from build123d import *

# Parameters (mm, degrees)
SKETCH_1_R      = 12
SKETCH_1_R_2    = 8
EXTRUDE_1_DEPTH = 6
SKETCH_2_W      = 18
SKETCH_2_H      = 2
EXTRUDE_2_DEPTH = 12


with BuildPart() as part:
    # 草图1 → 凸台-拉伸1 (new, symmetric)
    with BuildSketch(Plane.XY):
        Circle(SKETCH_1_R)
        Circle(SKETCH_1_R_2, mode=Mode.SUBTRACT)
    extrude(amount=EXTRUDE_1_DEPTH, both=True)

    # 草图2 → 凸台-拉伸2 (add)
    with BuildSketch(Plane.XY.offset(6)):
        with Locations((20.958260743, 0)):
            Rectangle(SKETCH_2_W, SKETCH_2_H)
    extrude(amount=-EXTRUDE_2_DEPTH)


solid = part.part
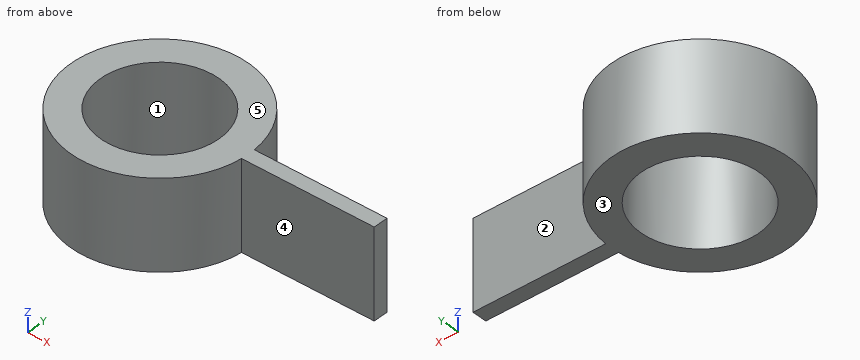
Part model, mm, in its own coordinate system. Face numbers are marked on the shaded views. A direction names the side the tool comes from. Give positions to 0.01 mm unless a question says otherwise; leave off trailing zeros. Order: outer loops, then holes, each group sorted by start corner. A loop starts at its lowest first (then second) coordinate and runs counter-clockwise, first axis right, second up. Notation, with made-up numbers: (-6.5, 45) - (6.5, 45) arc R15 cw to (6.5, 51) - close; hole circle Ø5 at (-23, -6). An arc over 180 degrees is marked (long way). Use a Markdown table: item, result.
1) 3-axis set-ups, long thin cutter, end or side, ignore diameter. For the marked faces 4 and 5: which of +Z, -Z, +X, -X, +Y, -Y reach the whole face in a straight line?
Checked values:
| item | result |
|---|---|
| face 4 | +Z, -Z, +X, -Y |
| face 5 | +Z, +X, -X, +Y, -Y |
2) Two-plate mould, pull along Y, no slides. Class the marked faces 1, 2 and 3: +Y half, -Y half, draft (parallel to the pull), parting line (faces both ways), or undercut.
Checked values:
| item | result |
|---|---|
| face 1 | undercut |
| face 2 | +Y half |
| face 3 | draft |
3) Flat gauge pins, fed straight in: P1, Ø6, axis at x = 21.5, z = 2.5, coming from the +Y side; P2, Ø3, axis at x = 12.5, z = -3.5, coming from the +Y side; P3, Ø3.5, axis at x = 19, z = 0, coming from the -Y side. Where does each tip first touch, or does it go through?
Checked values:
| item | result |
|---|---|
| P1 | y = 1 |
| P2 | y = 4.8 |
| P3 | y = -1 |
4) Saw through at A-A on y = 0. List the corners of the cut face in (x, z).
Checked values:
| item | result |
|---|---|
| outline | (-12, -6) - (-8, -6) - (-8, 6) - (-12, 6) - close; (8, -6) - (29.96, -6) - (29.96, 6) - (8, 6) - close |
5) Saw through at B-B on x = 0. List the corners of the cut face in (y, z).
Checked values:
| item | result |
|---|---|
| outline | (-12, -6) - (-8, -6) - (-8, 6) - (-12, 6) - close; (8, -6) - (12, -6) - (12, 6) - (8, 6) - close |
6) Probe L1, parallel to Y at x = 0, z = 2.25; L2, parallel to Y at x = 13, z = 4.5; L3, parallel to X at y = 4.25, z = -2.75. List the from-to ranges inside material, lowest first. Write a range as from..to.
Checked values:
| item | result |
|---|---|
| L1 | -12..-8, 8..12 |
| L2 | -1..1 |
| L3 | -11.22..-6.78, 6.78..11.22 |
7) Saw through at C-C on z = 1. List the corners of the cut face in (x, y).
Checked values:
| item | result |
|---|---|
| outline | (11.96, -1) - (29.96, -1) - (29.96, 1) - (11.96, 1) arc R12 ccw (long way) to start; hole circle Ø16 at (0, 0) |
8) Saw through at D-D on x = 14. List the corners of the cut face in (y, z), plus the area to 3 significant figures.
Checked values:
| item | result |
|---|---|
| outline | (-1, -6) - (1, -6) - (1, 6) - (-1, 6) - close |
| area | 24.0 mm² |
